Job drawing, mm, ordinate dimensions from the low corner. One solid piece. A direction names the side the tool comes from. Round coordinates to 2 decimals unless told otherwise and drop trailing zeros. Loops run counter-clockwise (first coordinate to the right, second up) from the corner with the lowest first, then second, coordinate; pieces in that order, holes last.
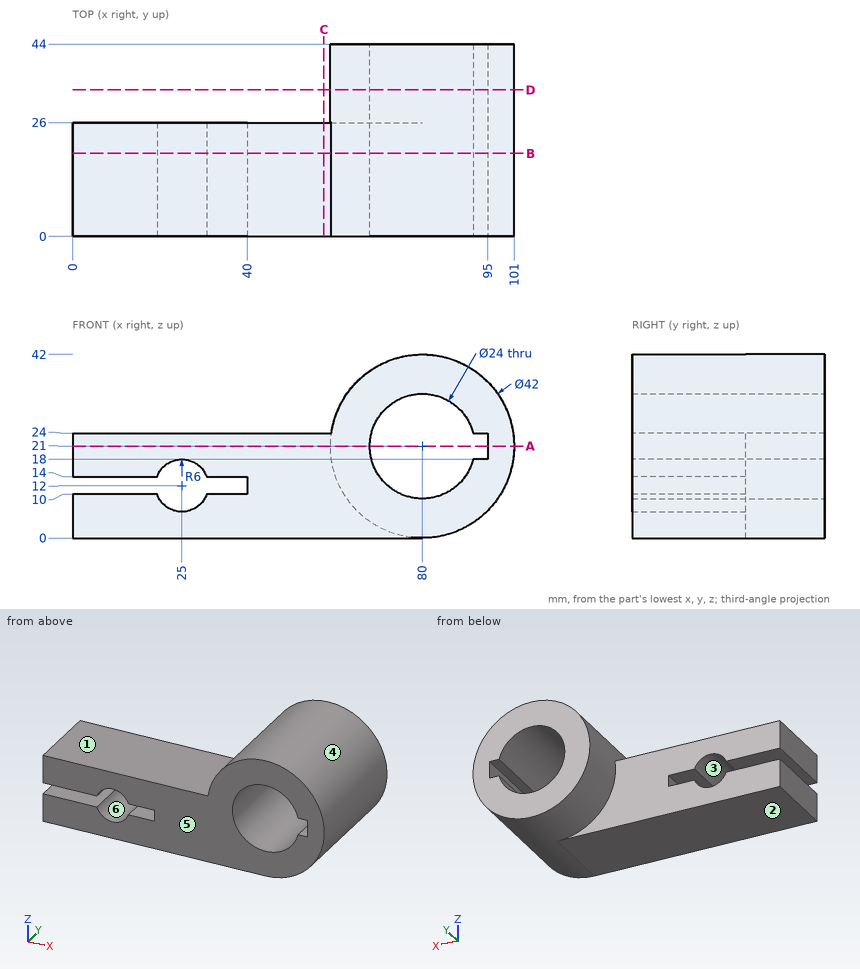
(1) Pin check, flat tips, straight feed: P1, Ø3, axis at y = 28, z = 20, coming from the -X side; P2, Ø21.5, axis at x = 7.5, y = 14.5, coming from the +Z side; P3, Ø1.7, axis at x = 93.5, y = 18, coming from the -Z side. Stop position of each tip, or through.
Responses:
P1: stops at x = 59
P2: stops at z = 24
P3: stops at z = 4.24
(2) Slice it at C-C on x = 57.5. List the corners of the cut face in (y, z).
Responses:
outline: (0, 0) - (26, 0) - (26, 24) - (0, 24) - close
(3) Slice it at A-A on z = 21. List the corners of the cut face in (x, y).
Responses:
outline: (0, 0) - (68, 0) - (68, 44) - (59, 44) - (59, 26) - (0, 26) - close; (95, 0) - (101, 0) - (101, 44) - (95, 44) - close
(4) Probe line 1 (X direction, y = 35.5, z = 21); line 2 (Z direction, x = 8, y = 3.5); line 3 (X direction, y = 3, z = 21). List the from-to ranges inside material, lowest first.
Responses:
line 1: x = 59 to 68, 95 to 101
line 2: z = 0 to 10, 14 to 24
line 3: x = 0 to 68, 95 to 101
(5) Which spindle directions (+Z, -Z, +X, -X, +Y, -Y) get a long thin tool onto all of the face, cutting with end or side? Do the marked faces 1, 2 and 3. Say none if no direction does.
Responses:
face 1: +Z, -X, +Y, -Y
face 2: -Z, +X, -X, +Y, -Y
face 3: +Y, -Y
(6) Slice it at B-B on y = 19. List the corners of the cut face in (x, z).
Responses:
outline: (0, 0) - (80, 0) arc R21 ccw (long way) to (59.22, 24) - (0, 24) - (0, 14) - (19.34, 14) arc R6 cw to (30.66, 14) - (40, 14) - (40, 10) - (30.66, 10) arc R6 cw to (19.34, 10) - (0, 10) - close; hole (91.62, 18) - (95, 18) - (95, 24) - (91.62, 24) arc R12 ccw (long way) to start
(7) Slice it at D-D on y = 33.5. List the corners of the cut face in (x, z).
Responses:
outline: circle Ø42 at (80, 21); hole (91.62, 18) - (95, 18) - (95, 24) - (91.62, 24) arc R12 ccw (long way) to start
(8) Pull direction X, two halves, no side cores. Call the marked faces 4, 5 and 6: +X half, -X half, draft (parallel to the pull), parting line (faces both ways), or undercut.
Responses:
face 4: parting line
face 5: draft
face 6: undercut
